Could you check a few things on this drawing? It's one solid part, dimensions in mm from its lowest x, y, z. A direction names the side the tool comes from. Round coordinates to 2 decimals unless told otherwise and drop trailing zeros. Loops run counter-clockwise (first coordinate to the right, second up) from the corner with the lowest first, then second, coordinate; pieces in that order, holes last. Notation, with made-up numbers: (22, -25) -> (78, -25) arc R21 ccw to (78, -12) -> close; hole circle Ø2 at (65, -38). An arc over 180 degrees is marked (long way). Write each question's results on one line, items separated by ' | '.
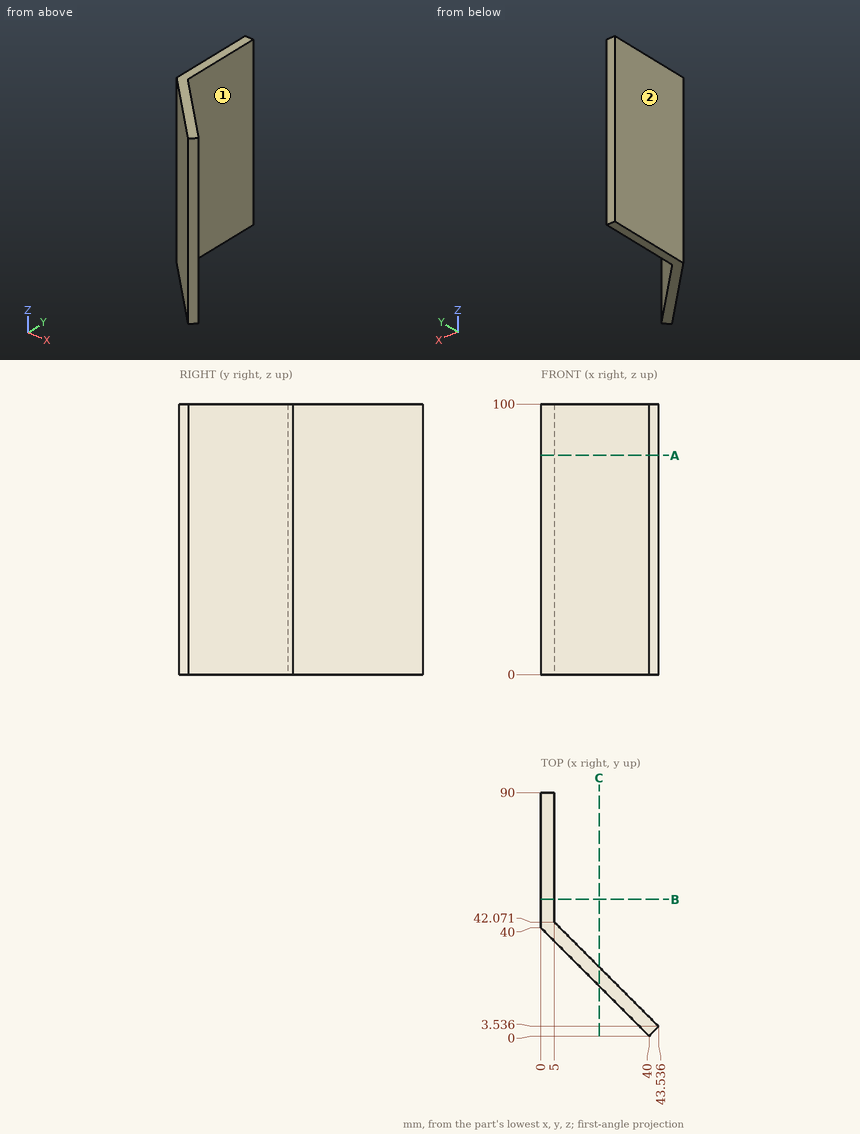
1) For the marked faces 1 and 2, which set-ups out of +Z, -Z, +X, -X, +Y, -Y let a thin tool reach every point of the face, with its end or its side?
Model answer:
face 1: +Z, -Z, +X, +Y | face 2: +Z, -Z, -X, +Y, -Y
2) I need wall thicknesses on line 1 (X direction, y = 68, z = 7); line 2 (Y direction, x = 38, z = 83.5); line 3 (X direction, y = 7, z = 67). Which ranges of each line are inside material? Lowest first, please.
Model answer:
line 1: x = 0 to 5 | line 2: y = 2 to 9.07 | line 3: x = 33 to 40.07
3) I want a section at A-A, the plane z = 81. Write out the boundary of the cut face in (x, y) (1 decimal).
Model answer:
outline: (0, 40) -> (40, 0) -> (43.5, 3.5) -> (5, 42.1) -> (5, 90) -> (0, 90) -> close
4) I'm going to push flat-ended pins straight in: pin 1 (14.5 mm diameter, centred on y = 56, z = 61.5, fed in from +X); pin 2 (3 mm diameter, centred on x = 27, z = 89, fed in from -Y). Where does each tip first touch, or does it pass through?
Model answer:
pin 1: stops at x = 5 | pin 2: stops at y = 11.5
5) I want a section at C-C, the plane x = 21.5. Write out the boundary of the cut face in (y, z), plus the area to 3 significant figures.
Model answer:
outline: (18.5, 0) -> (25.57, 0) -> (25.57, 100) -> (18.5, 100) -> close | area: 707 mm2
6) I want a section at B-B, the plane y = 50.5. Write out the boundary of the cut face in (x, z), plus the area to 3 significant figures.
Model answer:
outline: (0, 0) -> (5, 0) -> (5, 100) -> (0, 100) -> close | area: 500 mm2
